from build123d import *

# Parameters (mm, degrees)
BOSS_EXTRUDE1_DEPTH = 30
CUT_EXTRUDE1_DEPTH  = 25


with BuildPart() as part:
    # Sketch1 → Boss-Extrude1 (new body)
    with BuildSketch(Plane(origin=(0, 0, 0), x_dir=(1, 0, 0), z_dir=(0, 1, 0))):
        with BuildLine():
            Line((-220, 145), (220, 145))
            ThreePointArc((220, 145), (241.213203436, 136.213203436), (250, 115))
            Line((250, 115), (250, -115))
            ThreePointArc((250, -115), (241.213203436, -136.213203436), (220, -145))
            Line((220, -145), (-220, -145))
            ThreePointArc((-220, -145), (-241.213203436, -136.213203436), (-250, -115))
            Line((-250, -115), (-250, 115))
            ThreePointArc((-250, 115), (-241.213203436, 136.213203436), (-220, 145))
        make_face()
    extrude(amount=BOSS_EXTRUDE1_DEPTH)

    # Sketch2 → Cut-Extrude1 (cut)
    with BuildSketch(Plane(origin=(0, 30, 0), x_dir=(1, 0, 0), z_dir=(0, 1, 0))):
        with BuildLine():
            Line((-217, 142), (217, 142))
            ThreePointArc((217, 142), (238.213203436, 133.213203436), (247, 112))
            Line((247, 112), (247, -112))
            ThreePointArc((247, -112), (238.213203436, -133.213203436), (217, -142))
            Line((217, -142), (-217, -142))
            ThreePointArc((-217, -142), (-238.213203436, -133.213203436), (-247, -112))
            Line((-247, -112), (-247, 112))
            ThreePointArc((-247, 112), (-238.213203436, 133.213203436), (-217, 142))
        make_face()
    extrude(amount=-CUT_EXTRUDE1_DEPTH, mode=Mode.SUBTRACT)


solid = part.part
Input: part model. Units: mm. Frame: model coordinates. A direction names the side the tool comes from. Give positions to 0.01 mm unless a question says otherwise; leave off trailing zeros. Write each loop counter-clockwise with the first axis right and the second up, starting at its lowest first coordinate (ties: lowest second). Pieces come first, ordered by that corner, then holes.
Q1. Set-up query: faces 5 (the face through (238.445, 17.675, 132.979)), 6 (the face through (3, 0, -2)). Return all of +Z, -Z, +X, -X, +Y, -Y with unobstructed straight access to the full face (end or side cutting, diameter ignored); none if empty.
Q2. Pull-direction query (Z, two-part tool) for faces 1 (the face through (241.445, 14.79, 135.979)), 2 (the face through (-3, 18, -142)), 3 (the face through (-250, 15, 2)), 4 (the face through (240.979, 14.79, -136.445)); classes: pulls with the +Z half, pulls with the -Z half, needs draft (parallel to the pull), parting line crosses it, or undercut.
Q3. Material intervals for probe 1 along Z at (x, y) = (-97, 10.75); probe 2 along X at (y, z) = (6.75, 95); probe 3 along Y at (x, z) = (224.5, -91), sorted ascending.
Q4. First-contact query: P1, Ø3, axis at x = -154, z = -88, coming from the +Y side. Flat tip, straight axial feed; report the tip coordinate or a pass-through.
Q5. Section C-C, the plane x = -200.5. Output: boundary loops of the cut face in (y, z).
Q6. Section A-A, the plane y = 24.75. Output: boundary loops of the cut face in (x, z), plus the area to 3 significant figures.
Q7. Section B-B, the plane z = -50.5. Output: boundary loops of the cut face in (x, y), plus the area to 3 significant figures.
Filled in:
1. face 5: +Y
1. face 6: +Z, -Z, +X, -X, -Y
2. face 1: pulls with the +Z half
2. face 2: undercut
2. face 3: needs draft
2. face 4: pulls with the -Z half
3. probe 1: z = -145 to -142, 142 to 145
3. probe 2: x = -250 to -247, 247 to 250
3. probe 3: y = 0 to 5
4. P1: stops at y = 5
5. outline: (0, -145) - (30, -145) - (30, -142) - (5, -142) - (5, 142) - (30, 142) - (30, 145) - (0, 145) - close
6. outline: (-250, -115) arc R30 ccw to (-220, -145) - (220, -145) arc R30 ccw to (250, -115) - (250, 115) arc R30 ccw to (220, 145) - (-220, 145) arc R30 ccw to (-250, 115) - close; hole (-247, -112) arc R30 ccw to (-217, -142) - (217, -142) arc R30 ccw to (247, -112) - (247, 112) arc R30 ccw to (217, 142) - (-217, 142) arc R30 ccw to (-247, 112) - close
6. area: 4,700 mm2
7. outline: (-250, 0) - (250, 0) - (250, 30) - (247, 30) - (247, 5) - (-247, 5) - (-247, 30) - (-250, 30) - close
7. area: 2,650 mm2
